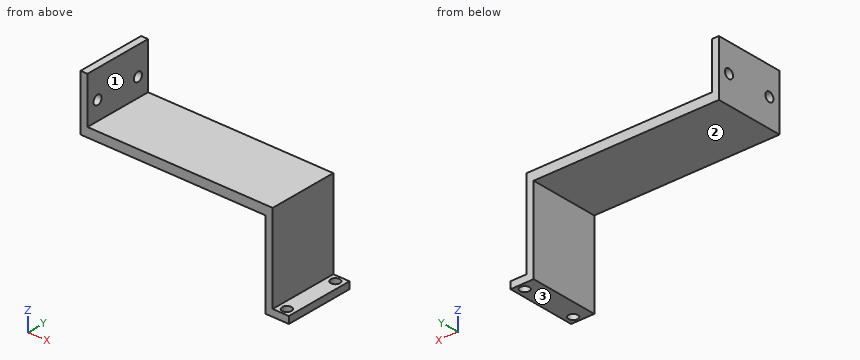
```python
from build123d import *

# Parameters (mm, degrees)
SKETCH_1_W          = 1.5
SKETCH_1_H          = 15
EXTRUDE_1_DEPTH     = 20.5
SKETCH_1_5_W        = 3.5
SKETCH_1_5_H        = 15
EXTRUDE_2_DEPTH     = 1.5
SKETCH_2_R          = 1
CUT_EXTRUDE_1_DEPTH = 1.5
SKETCH_3_W          = 2
SKETCH_3_H          = 15
EXTRUDE_3_DEPTH     = 40
SKETCH_4_W          = 1.5
SKETCH_4_H          = 15
EXTRUDE_4_DEPTH     = 10
SKETCH_5_R          = 1
CUT_EXTRUDE_3_DEPTH = 10


with BuildPart() as part:
    # 草图1 → 凸台-拉伸1 (new body)
    with BuildSketch(Plane.XY):
        with Locations((-1.75, 0)):
            Rectangle(SKETCH_1_W, SKETCH_1_H)
    extrude(amount=EXTRUDE_1_DEPTH)

    # 草图1<5> → 凸台-拉伸2 (add)
    with BuildSketch(Plane.XY):
        with Locations((0.75, 0)):
            Rectangle(SKETCH_1_5_W, SKETCH_1_5_H)
    extrude(amount=EXTRUDE_2_DEPTH)

    # 草图2 → 切除-拉伸1 (cut)
    with BuildSketch(Plane.XY.offset(1.5)):
        with Locations((0.75, 6)):
            Circle(SKETCH_2_R)
        with Locations((0.75, -6)):
            Circle(SKETCH_2_R)
    extrude(amount=-CUT_EXTRUDE_1_DEPTH, mode=Mode.SUBTRACT)

    # 草图3 → 凸台-拉伸3 (add)
    with BuildSketch(Plane.ZY.offset(2.5)):
        with Locations((19.5, 0)):
            Rectangle(SKETCH_3_W, SKETCH_3_H)
    extrude(amount=EXTRUDE_3_DEPTH)

    # 草图4 → 凸台-拉伸4 (add)
    with BuildSketch(Plane.XY.offset(20.5)):
        with Locations((-41.75, 0)):
            Rectangle(SKETCH_4_W, SKETCH_4_H)
    extrude(amount=EXTRUDE_4_DEPTH)

    # 草图5 → 切除-拉伸3 (cut)
    with BuildSketch(Plane.ZY.offset(42.5)):
        with Locations((24.5, 5)):
            Circle(SKETCH_5_R)
        with Locations((24.5, -5)):
            Circle(SKETCH_5_R)
    extrude(amount=-CUT_EXTRUDE_3_DEPTH, mode=Mode.SUBTRACT)


solid = part.part
```
Work out the finished part from the listing and answer in its coordinate system (mm). Face numbers are marked on the shaded views. A direction names the side the tool comes from. Round coordinates to 2 decimals unless told otherwise and drop trailing zeros. Loops run counter-clockwise (first coordinate to the right, second up) from the corner with the lowest first, then second, coordinate; pieces in that order, holes last.
(1) The part is cut by section A-A, the plane x = 0.75. Give the vertices of the cut face in (y, z).
Computed values:
outline: (-7.5, 0) - (-7, 0) - (-7, 1.5) - (-7.5, 1.5) - close; (-5, 0) - (5, 0) - (5, 1.5) - (-5, 1.5) - close; (7, 0) - (7.5, 0) - (7.5, 1.5) - (7, 1.5) - close
(2) Each of these flat-tipped pins is pushed along its axis until it touches: P1, Ø12, axis at x = -11, z = 3.5, coming from the -Y side; P2, Ø5, axis at y = 2.5, z = 26, coming from the +X side; P3, Ø12, axis at x = -29.5, z = 26, coming from the -Y side; P4, Ø1, axis at y = 2, z = 7.5, coming from the -X side. Where does it stop, or does it pass through?
Computed values:
P1: passes through
P2: stops at x = -41
P3: stops at y = -7.5
P4: stops at x = -2.5
(3) Find the intervals of material crossed by L1, parallel to Y at x = -41.65, z = 24.5; L2, parallel to Y at x = 0.75, z = 0.45; L3, parallel to X at y = 5.5, z = 28.5, in increasing order.
Computed values:
L1: y = -7.5 to -6, -4 to 4, 6 to 7.5
L2: y = -7.5 to -7, -5 to 5, 7 to 7.5
L3: x = -42.5 to -41
(4) The part is cut by section B-B, the plane z = 25. Give the vertices of the cut face in (x, y).
Computed values:
outline: (-42.5, -7.5) - (-41, -7.5) - (-41, -5.87) - (-42.5, -5.87) - close; (-42.5, -4.13) - (-41, -4.13) - (-41, 4.13) - (-42.5, 4.13) - close; (-42.5, 5.87) - (-41, 5.87) - (-41, 7.5) - (-42.5, 7.5) - close
(5) For the marked faces 1, 2 and 3, determine the directions among +Z, -Z, +X, -X, +Y, -Y from which every point of the face is accessible in a straight line to the end or side of a thin tool.
Computed values:
face 1: +Z, +X, +Y, -Y
face 2: -Z, -X, +Y, -Y
face 3: -Z, +X, -X, +Y, -Y
(6) The part is cut by section C-C, the plane x = -26. Give the vertices of the cut face in (y, z), and give its area (3 significant figures).
Computed values:
outline: (-7.5, 18.5) - (7.5, 18.5) - (7.5, 20.5) - (-7.5, 20.5) - close
area: 30.0 mm2
